Part model, mm, in its own coordinate system. A direction names the side the tool comes from. Give positions to 0.01 mm unless a question says otherwise; leave off trailing zeros. Write each loop counter-clockwise with the first axis right and the second up, starting at its lowest first coordinate (ties: lowest second). Pieces come first, ordered by that corner, then holes.
from build123d import *

# Parameters (mm, degrees)
SKETCH1_W           = 300
SKETCH1_H           = 200
BOSS_EXTRUDE1_DEPTH = 30


with BuildPart() as part:
    # Sketch1 → Boss-Extrude1 (new body)
    with BuildSketch(Plane.XY):
        with Locations((150, 100)):
            Rectangle(SKETCH1_W, SKETCH1_H)
        with BuildLine():
            Line((273.5, 130), (273.5, 70))
            ThreePointArc((273.5, 70), (260, 56.5), (246.5, 70))
            Line((246.5, 70), (246.5, 130))
            ThreePointArc((246.5, 130), (260, 143.5), (273.5, 130))
        make_face(mode=Mode.SUBTRACT)
        with BuildLine():
            Line((53.5, 130), (53.5, 70))
            ThreePointArc((53.5, 70), (40, 56.5), (26.5, 70))
            Line((26.5, 70), (26.5, 130))
            ThreePointArc((26.5, 130), (40, 143.5), (53.5, 130))
        make_face(mode=Mode.SUBTRACT)
    extrude(amount=BOSS_EXTRUDE1_DEPTH)


solid = part.part
1) 3-axis set-ups, long thin cutter, end or side, ignore diameter. For faces 1 (the flat face through (148, 101, 30)), 2 (the cylindrical face through (40.297, 56.503, 14.79)): which of +Z, -Z, +X, -X, +Y, -Y reach the whole face in a straight line?
Check result:
face 1: +Z, +X, -X, +Y, -Y
face 2: +Z, -Z
2) Saw through at B-B (x = 40). Write the cut outline in (y, z), and give its area (3 significant figures).
Check result:
outline: (0, 0) - (56.5, 0) - (56.5, 30) - (0, 30) - close; (143.5, 0) - (200, 0) - (200, 30) - (143.5, 30) - close
area: 3,390 mm2
3) Saw through at C-C (z = 4.5). Write the cut outline in (x, y), and give its area (3 significant figures).
Check result:
outline: (0, 0) - (300, 0) - (300, 200) - (0, 200) - close; hole (26.5, 70) arc R13.5 ccw to (53.5, 70) - (53.5, 130) arc R13.5 ccw to (26.5, 130) - close; hole (246.5, 70) arc R13.5 ccw to (273.5, 70) - (273.5, 130) arc R13.5 ccw to (246.5, 130) - close
area: 55,600 mm2
4) Drill centre lines: L1, parallel to X at y = 112, z = 5.5; L2, parallel to X at y = 137, z = 25.5. Where is each one in solid material? Low to high.
Check result:
L1: x = 0 to 26.5, 53.5 to 246.5, 273.5 to 300
L2: x = 0 to 28.46, 51.54 to 248.46, 271.54 to 300
5) Mould opens along Y. For faces 3 (the flat face through (300, 99, 15)), 4 (the cylindrical face through (259.703, 143.497, 14.79)), 5 (the flat face through (148, 0, 15)) say: +Y half, -Y half, draft (parallel to the pull), parting line (faces both ways), or undercut.
Check result:
face 3: draft
face 4: undercut
face 5: -Y half
6) Saw through at A-A (y = 123). Write the cut outline in (x, z), and give its area (3 significant figures).
Check result:
outline: (0, 0) - (26.5, 0) - (26.5, 30) - (0, 30) - close; (53.5, 0) - (246.5, 0) - (246.5, 30) - (53.5, 30) - close; (273.5, 0) - (300, 0) - (300, 30) - (273.5, 30) - close
area: 7,380 mm2
